```python
from build123d import *

# Parameters (mm, degrees)
SKETCH1_R           = 60
BOSS_EXTRUDE1_DEPTH = 10
FILLET2_R           = 1
SKETCH5_R           = 7.5
CUT_EXTRUDE2_DEPTH  = 86.440037535
SKETCH2_R           = 7.5
BOSS_EXTRUDE2_DEPTH = 10
BOSS_EXTRUDE4_DEPTH = 5


with BuildPart() as part:
    # Sketch1 → Boss-Extrude1 (new body)
    with BuildSketch(Plane(origin=(0, 0, 0), x_dir=(1, 0, 0), z_dir=(0, 1, 0))):
        with Locations(Location((0, 0, 0), (0, 0, 270))):
            Circle(SKETCH1_R)
    extrude(amount=BOSS_EXTRUDE1_DEPTH)

    # Fillet2
    fillet2_edges = [part.edges().sort_by_distance(p)[0] for p in [
        (0, 0, -60),
        (0, 10, -60),
    ]]
    fillet(fillet2_edges, radius=FILLET2_R)

    # Sketch5 → Cut-Extrude2 (cut, through all)
    with BuildSketch(Plane(origin=(0, 10, 0), x_dir=(1, 0, 0), z_dir=(0, 1, 0))):
        with Locations(Location((0, 0, 0), (0, 0, 270))):
            Circle(SKETCH5_R)
    cut_extrude2 = extrude(amount=-CUT_EXTRUDE2_DEPTH, mode=Mode.SUBTRACT)

    # Sketch2 → Boss-Extrude2 (add)
    with BuildSketch(Plane.XY.offset(47)):
        with BuildLine():
            Line((30, 0), (-30, 0))
            Line((-30, 0), (-30, -150))
            ThreePointArc((-30, -150), (0, -162.426406871), (30, -150))
            Line((30, -150), (30, 0))
        make_face()
        with Locations((0, -120)):
            Circle(SKETCH2_R, mode=Mode.SUBTRACT)
    boss_extrude2 = extrude(amount=BOSS_EXTRUDE2_DEPTH)

    # Sketch7 → Boss-Extrude4 (add)
    with BuildSketch(Plane.XY.offset(57)):
        with BuildLine():
            Line((-15.231546212, 0), (15.231546212, 0))
            Line((15.231546212, 0), (15.231546212, -33.694506244))
            ThreePointArc((15.231546212, -33.694506244), (15.147404529, -34.989015356), (14.896395444, -36.261740032))
            Line((14.896395444, -36.261740032), (7.393947913, -64.506158047))
            ThreePointArc((7.393947913, -64.506158047), (0, -70.192484331), (-7.393947913, -64.506158047))
            Line((-7.393947913, -64.506158047), (-14.896395444, -36.261740032))
            ThreePointArc((-14.896395444, -36.261740032), (-15.147404529, -34.989015356), (-15.231546212, -33.694506244))
            Line((-15.231546212, -33.694506244), (-15.231546212, 0))
        make_face()
    boss_extrude4 = extrude(amount=BOSS_EXTRUDE4_DEPTH)

    # Mirror2: Cut-Extrude2, Boss-Extrude2, Boss-Extrude4 across plane
    add(cut_extrude2.mirror(Plane.XY), mode=Mode.SUBTRACT)
    add(boss_extrude2.mirror(Plane.XY))
    add(boss_extrude4.mirror(Plane.XY))

    # Sketch10 → CBORE for M5 Hexagon head bolts-Full thread-grade C1 (revolve, cut)
    with BuildSketch(Plane(origin=(20, -150, -60), x_dir=(0, 1, 0), z_dir=(1, 0, 0))):
        Polygon((0, 0), (0, 122), (2.75, 122), (2.75, 0.5), (5.5, 0.5), (5.5, 0.025), (5.525, 0), align=None)
    cbore_for_m5_hexagon_head_bolts_full_thr = revolve(axis=Axis((20, -150, -66.35), (0, 0, 1)), mode=Mode.SUBTRACT)

    # Mirror3: CBORE for M5 Hexagon head bolts-Full thread-grade C1 across plane
    add(cbore_for_m5_hexagon_head_bolts_full_thr.mirror(Plane.ZY), mode=Mode.SUBTRACT)


solid = part.part
```
CAD build for the part. Positions are in the model's coordinates, mm. A direction names the side the tool comes from. Round coordinates to 2 decimals unless told otherwise and drop trailing zeros. Loops run counter-clockwise (first coordinate to the right, second up) from the corner with the lowest first, then second, coordinate; pieces in that order, holes last. Notation, with made-up numbers: M -19,29.5 L 18,29.5 A26 ccw 18,58.5 Z; hole C -36.75,36.25 d8. An arc over 180 degrees is marked long. Use a Markdown table: item, result. Add a question column.
(1) Pull direction Y, two halves, no side cores. Call faces 4 (the face through (0.14, -70.19, 59.46)), 5 (the face through (0, 0, 60)), 6 (the face through (-30, -74, -52)): +Y half, -Y half, draft (parallel to the pull), parting line (faces both ways), or undercut.
(2) Cut at B-B (z = 0). Give the cut face in (x, y).
(3) Which spindle directions (+Z, -Z, +X, -X, +Y, -Y) get a long thin tool onto all of the face, cutting with end or side? Do faces 1 (the face through (-11.093, -50.582, -59.465)), 2 (the face through (2.64, 4.94, -59.94)), 3 (the face through (11.198, -50.186, -59.465)). Say none if no direction does.
(4) Cut at A-A (x = 0). State how many separate pieces and enclosed holes the cut face has, and give its area (3 significant figures).
(5) Cut at C-C (y = -143). Give the cut face in (x, z), and give its area (3 significant figures).
(6) Drill centre lines: line 1 (X direction, y = -150, z = 50); line 2 (Z direction, x = 6.5, y = -68.5); line 3 (Z direction, x = -3.5, y = -3.5). Where is each one in solid material? Low to high.
(7) Cut at D-D (y = -117). Give the cut face in (x, z), and give its area (3 significant figures).
(8) Flat gauge pins, fed straight in: pin 1 (6.5 mm diameter, centred on x = -20, y = -150, fed in from -Z); pin 2 (10 mm diameter, centred on x = 38, z = -38, fed in from -Y); pin 3 (3.5 mm diameter, centred on x = 20, y = -150, fed in from -Z); pin 4 (5.5 mm diameter, centred on y = -22, z = -59.5, fed in from -X). Where does each tip first touch, or does it go through?
Geometry says:
| question | item | result |
|---|---|---|
| 1 | face 4 | -Y half |
| 1 | face 5 | undercut |
| 1 | face 6 | draft |
| 2 | outline | M -60,1 A1 ccw -59,0 L -7.5,0 L -7.5,10 L -59,10 A1 ccw -60,9 Z; M 7.5,0 L 59,0 A1 ccw 60,1 L 60,9 A1 ccw 59,10 L 7.5,10 Z |
| 3 | face 1 | -Z, -X, -Y |
| 3 | face 2 | +Y |
| 3 | face 3 | -Z, +X, -Y |
| 4 | separate pieces | 4 |
| 4 | enclosed holes | 0 |
| 4 | area | 4,700 mm² |
| 5 | outline | M -30,-57 L 30,-57 L 30,-47 L -30,-47 Z; M -30,47 L 30,47 L 30,57 L -30,57 Z |
| 5 | area | 1,200 mm² |
| 6 | line 1 | x = -30 to -22.75, -17.25 to 17.25, 22.75 to 30 |
| 6 | line 2 | z = -57 to -47, 47 to 57 |
| 6 | line 3 | z = -62 to -47, 47 to 62 |
| 7 | outline | M -30,-57 L -6.87,-57 L -6.87,-47 L -30,-47 Z; M -30,47 L -6.87,47 L -6.87,57 L -30,57 Z; M 6.87,-57 L 30,-57 L 30,-47 L 6.87,-47 Z; M 6.87,47 L 30,47 L 30,57 L 6.87,57 Z |
| 7 | area | 925 mm² |
| 8 | pin 1 | stops at z = -57 |
| 8 | pin 2 | stops at y = 0 |
| 8 | pin 3 | passes through |
| 8 | pin 4 | stops at x = -30 |
